Could you check a few things on this model? Use its own coordinates, in mm. A direction names the side the tool comes from. Coordinates: 2 decimals unless noted, no trailing zeros. Order: outer loops, then holes, each group sorted by start corner. A loop starts at its lowest first (then second) coordinate and runs counter-clockwise, first axis right, second up.
```python
from build123d import *

# Parameters (mm, degrees)
SKETCH1_W                    = 30
SKETCH1_H                    = 74
SKETCH1_R                    = 11
BOSS_EXTRUDE1_DEPTH          = 10
SKETCH3_W                    = 15
SKETCH3_H                    = 10
BOSS_EXTRUDE2_DEPTH          = 8
SKETCH4_R                    = 2.75
CUT_EXTRUDE1_DEPTH           = 71.576199954
F_4_0_4_DIAMETER_HOLE1_D     = 4
F_4_0_4_DIAMETER_HOLE1_DEPTH = 10
F_4_0_4_DIAMETER_HOLE1_TIP   = 1.201721238
CHAMFER1_SIZE                = 5
CHAMFER2_SIZE                = 1


with BuildPart() as part:
    # Sketch1 → Boss-Extrude1 (new body)
    with BuildSketch(Plane.XY):
        with Locations((0, 37)):
            Rectangle(SKETCH1_W, SKETCH1_H)
        with Locations((0, 60)):
            Circle(SKETCH1_R, mode=Mode.SUBTRACT)
    extrude(amount=BOSS_EXTRUDE1_DEPTH)

    # Sketch3 → Boss-Extrude2 (add)
    with BuildSketch(Plane.XZ):
        with Locations((-7.5, 15)):
            Rectangle(SKETCH3_W, SKETCH3_H)
        with Locations((7.5, 15)):
            Rectangle(SKETCH3_W, SKETCH3_H)
    extrude(amount=-BOSS_EXTRUDE2_DEPTH)

    # Sketch4 → Cut-Extrude1 (cut, through all)
    with BuildSketch(Plane(origin=(0, 8, 0), x_dir=(-1, 0, 0), z_dir=(0, 1, 0))):
        with Locations((10, 15)):
            Circle(SKETCH4_R)
        with Locations(Location((-10, 15, 0), (0, 0, 180))):
            Circle(SKETCH4_R)
    extrude(amount=-CUT_EXTRUDE1_DEPTH, mode=Mode.SUBTRACT)

    # Ø4.0 (4) Diameter Hole1
    with Locations(Plane.XZ):
        with Locations((-10, 5), (10, 5)):
            Hole(F_4_0_4_DIAMETER_HOLE1_D / 2, depth=F_4_0_4_DIAMETER_HOLE1_DEPTH)
            with Locations((0, 0, -(F_4_0_4_DIAMETER_HOLE1_DEPTH + F_4_0_4_DIAMETER_HOLE1_TIP / 2))):  # 118° drill point
                Cone(0, F_4_0_4_DIAMETER_HOLE1_D / 2, F_4_0_4_DIAMETER_HOLE1_TIP, mode=Mode.SUBTRACT)

    # Chamfer1
    chamfer1_edges = [part.edges().sort_by_distance(p)[0] for p in [
        (-15, 74, 5),
        (15, 74, 5),
    ]]
    chamfer(chamfer1_edges, length=CHAMFER1_SIZE)

    # Chamfer2
    chamfer2_edges = [part.edges().sort_by_distance(p)[0] for p in [
        (-15, 4, 20),
        (15, 4, 20),
        (0, 0, 0),
    ]]
    chamfer(chamfer2_edges, length=CHAMFER2_SIZE)


solid = part.part
```
Item 1: I need wall thicknesses on line 1 (X direction, y = 3.25, z = 5); line 2 (Z direction, x = -10, y = 4.75); line 3 (Z direction, x = 12.75, y = 51.5). Which ranges of each line are inside material? Lowest first, please.
Item 2: Suppose I cut it at D-D (y = 26.5). List the corners of the cut face in (x, z) for me, and give its area (3 significant figures).
Item 3: For pin 1 Ø10 at (x, z) = (4, 8.5) entering from -Y; pin 2 Ø3 at (x, z) = (-6, 15) entering from +Y, each with a flat end and sliding along its axis, tell me the tip position at first contact or that it passes through.
Item 4: Thinking about a two-plate mould opening in X: for faces 1 (the face through (-1.432, 70.906, 4.93)), 2 (the face through (-9.642, 4.056, 17.727)), 3 (the face through (-15, 34, 5)), 4 (the face through (0, 4, 20)), which applies, +X half, -X half, draft (parallel to the pull), parting line (faces both ways), or undercut?
Item 5: Suppose I cut it at C-C (x = 3). List the corners of the cut face in (y, z) for me.
Item 6: Suppose I cut it at B-B (z = 15). List the corners of the cut face in (x, y) for me, and give its area (3 significant figures).
Item 7: Which directions (+Z, -Z, +X, -X, +Y, -Y) give clear straight access to the entire face, cutting with the end or side of a thin tool? Please do faces 5 (the face through (0, 34, 10)), 6 (the face through (0, 30, 0)), 7 (the face through (12, 5, 5)).
Item 8: Suppose I cut it at A-A (x = 0). List the corners of the cut face in (y, z) for me.
Geometry results:
1. line 1: x = -15 to -12, -8 to 8, 12 to 15
1. line 2: z = 0 to 3, 7 to 12.25, 17.75 to 20
1. line 3: z = 0 to 10
2. outline: (-15, 0) - (15, 0) - (15, 10) - (-15, 10) - close
2. area: 300 mm2
3. pin 1: stops at y = 0
3. pin 2: stops at y = 8
4. face 1: undercut
4. face 2: undercut
4. face 3: -X half
4. face 4: draft
5. outline: (0, 1) - (1, 0) - (49.42, 0) - (49.42, 10) - (8, 10) - (8, 20) - (0, 20) - close; (70.58, 0) - (74, 0) - (74, 10) - (70.58, 10) - close
6. outline: (-15, 0) - (-12.75, 0) - (-12.75, 8) - (-15, 8) - close; (-7.25, 0) - (7.25, 0) - (7.25, 8) - (-7.25, 8) - close; (12.75, 0) - (15, 0) - (15, 8) - (12.75, 8) - close
6. area: 152 mm2
7. face 5: +Z, +X, -X, +Y
7. face 6: -Z, +X, -X, +Y, -Y
7. face 7: -Y
8. outline: (0, 1) - (1, 0) - (49, 0) - (49, 10) - (8, 10) - (8, 20) - (0, 20) - close; (71, 0) - (74, 0) - (74, 10) - (71, 10) - close
